For this review, take the finished solid that the model builds, in its own axes (mm). Face numbers are marked on the shaded views. Round coordinates to 2 decimals unless told otherwise and drop trailing zeros. Order: outer loops, then holes, each group sorted by start corner. A loop starts at its lowest first (then second) coordinate and runs counter-clockwise, first axis right, second up. Notation, with made-up numbers: (-0.75, 37) -> (26.25, 37) arc R21 ccw to (26.25, 44) -> close; hole circle Ø6 at (84.5, -38.75). An arc over 180 degrees is marked (long way). Use a Markdown table: item, result. Add a question column.
1) Draft analysis for pull direction Z (two halves, no side actions). For the marked faces 1, 2, 3 and 4, state which applies: pulls with the +Z half, pulls with the -Z half, needs draft (parallel to the pull), parting line crosses it, or undercut.
2) Wall thickness on line 1 along Y through (x, z) = (0, -3.65); line 2 along Z through (x, y) = (0, 7); line 3 along X through (y, z) = (11, 0): over which ranges is each line inside the solid? List them lowest first. Write a range as [from, to].
3) Clearance check with flat-ended pins moving along their axes: P1, Ø3, axis at y = 12, z = -2, coming from the -X side; P2, Ø2, axis at y = 10, z = -2, coming from the -X side. State where each tip first meets the part, or that it passes through.
4) Consider section D-D (x = 0.5). State the section outline as (y, z) points, plus the area to 3 significant figures.
5) Consider section C-C (x = 2.5). State the section outline as (y, z) points.
6) Consider section B-B (y = 10). State the section outline as (x, z) points.
7) Consider section A-A (z = 0). State the section outline as (x, y) points, plus the area to 3 significant figures.
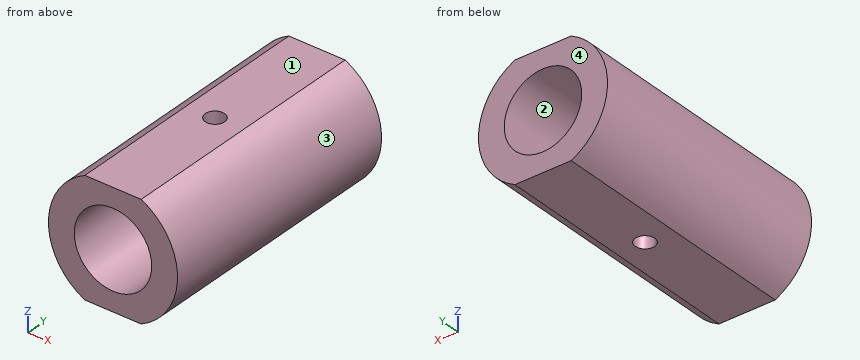
```python
from build123d import *

# Parameters (mm, degrees)
SKETCH1_R           = 3
BOSS_EXTRUDE1_DEPTH = 20
SKETCH2_R           = 0.75
CUT_EXTRUDE1_DEPTH  = 20


with BuildPart() as part:
    # Sketch1 → Boss-Extrude1 (new body)
    with BuildSketch(Plane(origin=(0, 0, 0), x_dir=(1, 0, 0), z_dir=(0, 1, 0))):
        with BuildLine():
            Line((2.179449472, -4.5), (-2.179449472, -4.5))
            ThreePointArc((-2.179449472, -4.5), (-5, 0), (-2.179449472, 4.5))
            Line((-2.179449472, 4.5), (2.179449472, 4.5))
            ThreePointArc((2.179449472, 4.5), (5, 0), (2.179449472, -4.5))
        make_face()
        with Locations(Location((0, 0, 0), (0, 0, 270))):
            Circle(SKETCH1_R, mode=Mode.SUBTRACT)
    extrude(amount=BOSS_EXTRUDE1_DEPTH)

    # Sketch2 → Cut-Extrude1 (cut)
    with BuildSketch(Plane(origin=(0, 0, -4.5), x_dir=(-1, 0, 0), z_dir=(0, 0, -1))):
        with Locations((0, 10)):
            Circle(SKETCH2_R)
    extrude(amount=-CUT_EXTRUDE1_DEPTH, mode=Mode.SUBTRACT)


solid = part.part
```
Results list:
| question | item | result |
|---|---|---|
| 1 | face 1 | pulls with the +Z half |
| 1 | face 2 | undercut |
| 1 | face 3 | parting line crosses it |
| 1 | face 4 | needs draft |
| 2 | line 1 | [0, 9.25], [10.75, 20] |
| 2 | line 2 | [-4.5, -3], [3, 4.5] |
| 2 | line 3 | [-5, -3], [3, 5] |
| 3 | P1 | x = -4.97 |
| 3 | P2 | x = -4.9 |
| 4 | outline | (0, -4.5) -> (9.44, -4.5) -> (9.44, -2.96) -> (0, -2.96) -> close; (0, 2.96) -> (9.44, 2.96) -> (9.44, 4.5) -> (0, 4.5) -> close; (10.56, -4.5) -> (20, -4.5) -> (20, -2.96) -> (10.56, -2.96) -> close; (10.56, 2.96) -> (20, 2.96) -> (20, 4.5) -> (10.56, 4.5) -> close |
| 4 | area | 58.2 mm2 |
| 5 | outline | (0, -4.33) -> (20, -4.33) -> (20, -1.66) -> (0, -1.66) -> close; (0, 1.66) -> (20, 1.66) -> (20, 4.33) -> (0, 4.33) -> close |
| 6 | outline | (-2.18, -4.5) -> (-0.75, -4.5) -> (-0.75, -2.9) arc R3 cw to (-0.75, 2.9) -> (-0.75, 4.5) -> (-2.18, 4.5) arc R5 ccw to start; (0.75, -4.5) -> (2.18, -4.5) arc R5 ccw to (2.18, 4.5) -> (0.75, 4.5) -> (0.75, 2.9) arc R3 cw to (0.75, -2.9) -> close |
| 7 | outline | (-5, 0) -> (-3, 0) -> (-3, 20) -> (-5, 20) -> close; (3, 0) -> (5, 0) -> (5, 20) -> (3, 20) -> close |
| 7 | area | 80.0 mm2 |
